CAD build for the part. Positions are in the model's coordinates, mm. Give positions to 0.01 mm unless a question says otherwise; leave off trailing zeros. Write each loop counter-clockwise with the first axis right and the second up, starting at its lowest first coordinate (ties: lowest second). Pieces come first, ordered by that corner, then holes. Notation, with made-up numbers: (16.25, 62.25) - (50.25, 62.25) arc R13 ccw to (50.25, 77.25) - close; hole circle Ø10 at (-1.75, -38.75). An arc over 180 degrees is marked (long way). Write item = value, one per line. Start each with the question number.
```python
from build123d import *

# Parameters (mm, degrees)
SKETCH_1_W                = 210
SKETCH_1_H                = 10
EXTRUDE_1_DEPTH           = 12.5
HOLE_WIZARD_1_D           = 4.5
HOLE_WIZARD_1_CBORE_D     = 8
HOLE_WIZARD_1_CBORE_DEPTH = 5
SKETCH_5_R                = 3
CUT_EXTRUDE_1_DEPTH       = 29


with BuildPart() as part:
    # 草图1 → 凸台-拉伸1 (new, symmetric)
    with BuildSketch(Plane(origin=(0, 0, 0), x_dir=(0, 0, -1), z_dir=(1, 0, 0))):
        Rectangle(SKETCH_1_W, SKETCH_1_H)
    extrude(amount=EXTRUDE_1_DEPTH, both=True)

    # 打孔尺寸(%根据)开槽圆柱头螺钉的类型1 (through all)
    with Locations(Plane.ZY.offset(12.5)):
        with Locations((0, 0), (-75, 0), (75, 0)):
            CounterBoreHole(HOLE_WIZARD_1_D / 2, HOLE_WIZARD_1_CBORE_D / 2, HOLE_WIZARD_1_CBORE_DEPTH)

    # 草图5 → 切除-拉伸1 (cut)
    with BuildSketch(Plane.XZ.offset(5)):
        with Locations(Location((0, 50.563507408, 0), (0, 0, 270))):
            Circle(SKETCH_5_R)
        with Locations(Location((0, -49.436492592, 0), (0, 0, 270))):
            Circle(SKETCH_5_R)
    extrude(amount=-CUT_EXTRUDE_1_DEPTH, mode=Mode.SUBTRACT)


solid = part.part
```
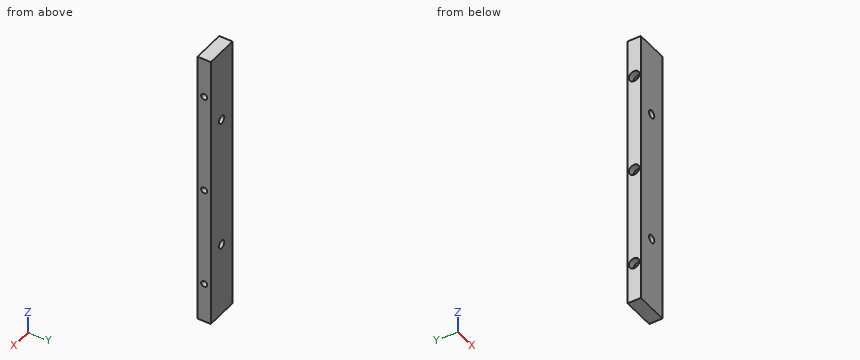
1. Wall check: line 1 along X through (y, z) = (0, 52.5); line 2 along Z through (x, y) = (9.5, 2); line 3 along Z through (x, y) = (-10.75, 2.25). Give the ranges that are in metal, low to high.
2. Cut at D-D (x = -10). Give the cut face in (y, z), then the cut area to 3 significant figures.
3. Pin check, flat tips, straight feed: pin 1 Ø2.5 at (y, z) = (0, -75) entering from +X; pin 2 Ø4 at (y, z) = (-1, 75.5) entering from -X. Stop position of each tip, or through.
4. Cut at A-A (x = 0). Give the cut face in (y, z), then the cut area to 3 significant figures.
5. Cut at C-C (z = -75). Give the cut face in (x, y).
6. Cut at B-B (y = 0). Count the separate pieces of the cut face and the enclosed holes in it, then the cut area to 3 significant figures.
Output:
q1.line_1 = -12.5 to -2.29, 2.29 to 12.5
q1.line_2 = -105 to -76.03, -73.97 to -1.03, 1.03 to 73.97, 76.03 to 105
q1.line_3 = -105 to -78.31, -71.69 to -3.31, 3.31 to 71.69, 78.31 to 105
q2.outline = (-5, -105) - (5, -105) - (5, 105) - (-5, 105) - close; hole circle Ø8 at (0, -75); hole circle Ø8 at (0, 0); hole circle Ø8 at (0, 75)
q2.area = 1,950 mm2
q3.pin_1 = through
q3.pin_2 = -7.5
q4.outline = (-5, -105) - (5, -105) - (5, -52.44) - (-5, -52.44) - close; (-5, -46.44) - (5, -46.44) - (5, 47.56) - (-5, 47.56) - close; (-5, 53.56) - (5, 53.56) - (5, 105) - (-5, 105) - close; hole circle Ø4.5 at (0, -75); hole circle Ø4.5 at (0, 0); hole circle Ø4.5 at (0, 75)
q4.area = 1,930 mm2
q5.outline = (-12.5, -5) - (12.5, -5) - (12.5, -2.25) - (-7.5, -2.25) - (-7.5, -4) - (-12.5, -4) - close; (-12.5, 4) - (-7.5, 4) - (-7.5, 2.25) - (12.5, 2.25) - (12.5, 5) - (-12.5, 5) - close
q6.separate_pieces = 4
q6.enclosed_holes = 2
q6.area = 4,800 mm2
